Source: CAD feature listing. Evaluate the final solid. Frame: model axes, mm. Give positions to 0.01 mm unless a question says otherwise; leave off trailing zeros. Write each loop counter-clockwise with the first axis right and the second up, starting at its lowest first coordinate (ties: lowest second). Pieces come first, ordered by that corner, then holes. Notation, with made-up numbers: (-21.75, 23) -> (-11.75, 23) arc R22 cw to (-11.75, 55) -> close; hole circle Ø5 at (-2, 20.25). An arc over 180 degrees is marked (long way). Write item = value, one per line.
from build123d import *

# Parameters (mm, degrees)
SKETCH_1_W                                         = 130
SKETCH_1_H                                         = 230
BOSS_EXTRUDE_1_DEPTH                               = 10
M6_TAPPED_HOLE_1_D                                 = 5
LINEAR_PATTERN_1_COUNT                             = 2
LINEAR_PATTERN_1_PITCH                             = 15
M5_SOCKET_HEAD_CAP_SCREW_COUNTERBORE_1_D           = 5.5
M5_SOCKET_HEAD_CAP_SCREW_COUNTERBORE_1_CBORE_D     = 10
M5_SOCKET_HEAD_CAP_SCREW_COUNTERBORE_1_CBORE_DEPTH = 5
LINEAR_PATTERN_2_COUNT                             = 3
LINEAR_PATTERN_2_PITCH                             = 50
LINEAR_PATTERN_2_COL_COUNT                         = 3
LINEAR_PATTERN_2_COL_PITCH                         = 50
LINEAR_PATTERN_3_COUNT                             = 2
LINEAR_PATTERN_3_PITCH                             = 110
LINEAR_PATTERN_3_COPY_1_D                          = 5
LINEAR_PATTERN_4_COUNT                             = 2
LINEAR_PATTERN_4_PITCH                             = 215
LINEAR_PATTERN_4_COPY_1_D                          = 5
CUT_EXTRUDE_1_DEPTH                                = 133.476412995
LINEAR_PATTERN_8_COUNT                             = 3
LINEAR_PATTERN_8_PITCH                             = 60
LINEAR_PATTERN_7_COUNT                             = 2
LINEAR_PATTERN_7_PITCH                             = 40
LINEAR_PATTERN_7_COPY_1_D                          = 5


with BuildPart() as part:
    # Sketch 1 → Boss-Extrude 1 (new body)
    with BuildSketch(Plane(origin=(0, 0, 0), x_dir=(0, 0, -1), z_dir=(1, 0, 0))):
        Rectangle(SKETCH_1_W, SKETCH_1_H)
    extrude(amount=BOSS_EXTRUDE_1_DEPTH)

    # M6 Tapped Hole 1 (through all)
    with Locations(Plane.ZY):
        with Locations((12, -107.5)):
            m6_tapped_hole_1 = Hole(M6_TAPPED_HOLE_1_D / 2)

    # Linear Pattern 1: M6 Tapped Hole 1 ×2
    with Locations(*[(0, 0, -i * LINEAR_PATTERN_1_PITCH) for i in range(1, LINEAR_PATTERN_1_COUNT)]):
        add(m6_tapped_hole_1, mode=Mode.SUBTRACT)

    # M5 Socket Head Cap Screw Counterbore 1 (through all)
    with Locations(Plane(origin=(10, 0, 0), x_dir=(0, 0, -1), z_dir=(1, 0, 0))):
        with Locations((59, 0)):
            m5_socket_head_cap_screw_counterbore_1 = CounterBoreHole(M5_SOCKET_HEAD_CAP_SCREW_COUNTERBORE_1_D / 2, M5_SOCKET_HEAD_CAP_SCREW_COUNTERBORE_1_CBORE_D / 2, M5_SOCKET_HEAD_CAP_SCREW_COUNTERBORE_1_CBORE_DEPTH)

    # Linear Pattern 2: M5 Socket Head Cap Screw Counterbore 1 ×3
    with Locations(*[(0, i * LINEAR_PATTERN_2_PITCH, 0) for i in range(1, LINEAR_PATTERN_2_COUNT)]):
        add(m5_socket_head_cap_screw_counterbore_1, mode=Mode.SUBTRACT)

    # Linear Pattern 2 col: M5 Socket Head Cap Screw Counterbore 1 ×3
    with Locations(*[(0, -i * LINEAR_PATTERN_2_COL_PITCH, 0) for i in range(1, LINEAR_PATTERN_2_COL_COUNT)]):
        add(m5_socket_head_cap_screw_counterbore_1, mode=Mode.SUBTRACT)

    # Linear Pattern 3: M6 Tapped Hole 1 ×2
    with Locations(*[(0, i * LINEAR_PATTERN_3_PITCH, 0) for i in range(1, LINEAR_PATTERN_3_COUNT)]):
        add(m6_tapped_hole_1, mode=Mode.SUBTRACT)

    # Linear Pattern 3 copy 1 (through all)
    with Locations(Plane(origin=(0, 110, -15), x_dir=(0, 0, 1), z_dir=(-1, 0, 0))):
        with Locations((12, -107.5)):
            Hole(LINEAR_PATTERN_3_COPY_1_D / 2)

    # Linear Pattern 4: M6 Tapped Hole 1 ×2
    with Locations(*[(0, i * LINEAR_PATTERN_4_PITCH, 0) for i in range(1, LINEAR_PATTERN_4_COUNT)]):
        add(m6_tapped_hole_1, mode=Mode.SUBTRACT)

    # Linear Pattern 4 copy 1 (through all)
    with Locations(Plane(origin=(0, 215, -15), x_dir=(0, 0, 1), z_dir=(-1, 0, 0))):
        with Locations((12, -107.5)):
            Hole(LINEAR_PATTERN_4_COPY_1_D / 2)

    # Sketch 8 → Cut-Extrude 1 (cut, through all)
    with BuildSketch(Plane.ZY):
        with BuildLine():
            Line((-36, -81.7), (46, -81.7))
            ThreePointArc((46, -81.7), (49.3, -85), (46, -88.3))
            Line((46, -88.3), (-36, -88.3))
            ThreePointArc((-36, -88.3), (-39.3, -85), (-36, -81.7))
        make_face()
    cut_extrude_1 = extrude(amount=-CUT_EXTRUDE_1_DEPTH, mode=Mode.SUBTRACT)

    # Linear Pattern 8: Cut-Extrude 1 ×3
    with Locations(*[(0, i * LINEAR_PATTERN_8_PITCH, 0) for i in range(1, LINEAR_PATTERN_8_COUNT)]):
        add(cut_extrude_1, mode=Mode.SUBTRACT)

    # Linear Pattern 7: M6 Tapped Hole 1 ×2
    with Locations(*[(0, i * LINEAR_PATTERN_7_PITCH, 0) for i in range(1, LINEAR_PATTERN_7_COUNT)]):
        add(m6_tapped_hole_1, mode=Mode.SUBTRACT)

    # Linear Pattern 7 copy 1 (through all)
    with Locations(Plane(origin=(0, 40, -15), x_dir=(0, 0, 1), z_dir=(-1, 0, 0))):
        with Locations((12, -107.5)):
            Hole(LINEAR_PATTERN_7_COPY_1_D / 2)


solid = part.part
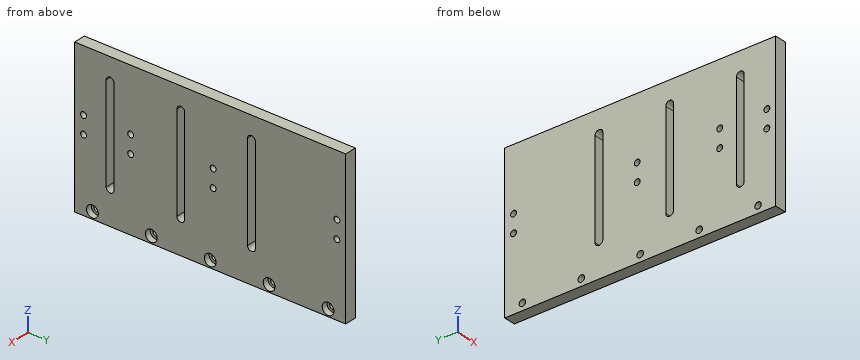
1) Cut plane D-D (y = -85). Return the cut outline in (x, z), then the cut area to 3 significant figures.
Computed:
outline = (0, -65) -> (10, -65) -> (10, -39.3) -> (0, -39.3) -> close; (0, 49.3) -> (10, 49.3) -> (10, 65) -> (0, 65) -> close
area = 414 mm²
2) Cut plane C-C (x = 2.5). State how many separate pieces and enclosed holes the cut face has, then the cut area to 3 significant figures.
Computed:
separate_pieces = 1
enclosed_holes = 16
area = 27,900 mm²
3) Contact query for a flat-ended pin moving along its axis: pin 1 (5 mm diameter, centred on y = -51, z = -58.5, fed in from +X). Output: stop coordinate, or through.
Computed:
pin_1 = 5
4) Cut plane A-A (y = 107.5). Return the cut outline in (x, z).
Computed:
outline = (0, -65) -> (10, -65) -> (10, -5.5) -> (0, -5.5) -> close; (0, -0.5) -> (10, -0.5) -> (10, 9.5) -> (0, 9.5) -> close; (0, 14.5) -> (10, 14.5) -> (10, 65) -> (0, 65) -> close
5) Material intervals for L1, parallel to Y at x = 7.15, z = -59; L2, parallel to Y at x = 6, z = 33.5; L3, parallel to Y at x = 1.5, z = -37, sorted ascending.
Computed:
L1 = -115 to -105, -95 to -55, -45 to -5, 5 to 45, 55 to 95, 105 to 115
L2 = -115 to -88.3, -81.7 to -28.3, -21.7 to 31.7, 38.3 to 115
L3 = -115 to -88.14, -81.86 to -28.14, -21.86 to 31.86, 38.14 to 115
6) Cut plane B-B (z = -26.5). Return the cut outline in (x, y).
Computed:
outline = (0, -115) -> (10, -115) -> (10, -88.3) -> (0, -88.3) -> close; (0, -81.7) -> (10, -81.7) -> (10, -28.3) -> (0, -28.3) -> close; (0, -21.7) -> (10, -21.7) -> (10, 31.7) -> (0, 31.7) -> close; (0, 38.3) -> (10, 38.3) -> (10, 115) -> (0, 115) -> close
